CAD build for the part. Positions are in the model's coordinates, mm. Face numbers are marked on the shaded views. A direction names the side the tool comes from. Give positions to 0.01 mm unless a question says otherwise; leave off trailing zeros. Loops run counter-clockwise (first coordinate to the right, second up) from the corner with the lowest first, then second, coordinate; pieces in that order, holes last. Notation, with made-up numbers: (69.5, 53) -> (117.5, 53) arc R29 cw to (117.5, 76) -> close; hole circle Ø7 at (-13.5, 81). An arc over 180 degrees is marked (long way). Use one line per item in the form item = value.
```python
from build123d import *

# Parameters (mm, degrees)
SKETCH1_R           = 12.5
BOSS_EXTRUDE1_DEPTH = 3
SKETCH2_R           = 12
BOSS_EXTRUDE2_DEPTH = 25
SKETCH3_R           = 7.5
BOSS_EXTRUDE3_DEPTH = 12
CUT_EXTRUDE1_DEPTH  = 4
CHAMFER1_SIZE       = 1


with BuildPart() as part:
    # Sketch1 → Boss-Extrude1 (new body)
    with BuildSketch(Plane(origin=(0, 0, 0), x_dir=(1, 0, 0), z_dir=(0, 1, 0))):
        with Locations(Location((0, 0, 0), (0, 0, 270))):
            Circle(SKETCH1_R)
    extrude(amount=BOSS_EXTRUDE1_DEPTH)

    # Sketch2 → Boss-Extrude2 (add)
    with BuildSketch(Plane(origin=(0, 3, 0), x_dir=(1, 0, 0), z_dir=(0, 1, 0))):
        with Locations(Location((0, 0, 0), (0, 0, 270))):
            Circle(SKETCH2_R)
    extrude(amount=BOSS_EXTRUDE2_DEPTH)

    # Sketch3 → Boss-Extrude3 (add)
    with BuildSketch(Plane(origin=(0, 28, 0), x_dir=(1, 0, 0), z_dir=(0, 1, 0))):
        with Locations(Location((0, 0, 0), (0, 0, 270))):
            Circle(SKETCH3_R)
    extrude(amount=BOSS_EXTRUDE3_DEPTH)

    # Sketch4 → Cut-Extrude1 (cut)
    with BuildSketch(Plane(origin=(0, 0, -12), x_dir=(-1, 0, 0), z_dir=(0, 0, -1))):
        with BuildLine():
            Line((4, 23), (4, 8))
            ThreePointArc((4, 8), (0, 4), (-4, 8))
            Line((-4, 8), (-4, 23))
            ThreePointArc((-4, 23), (0, 27), (4, 23))
        make_face()
    extrude(amount=-CUT_EXTRUDE1_DEPTH, mode=Mode.SUBTRACT)

    # Chamfer1
    chamfer1_edges = [part.edges().sort_by_distance(p)[0] for p in [
        (0, 40, -7.5),
        (0, 0, -12.5),
    ]]
    chamfer(chamfer1_edges, length=CHAMFER1_SIZE)


solid = part.part
```
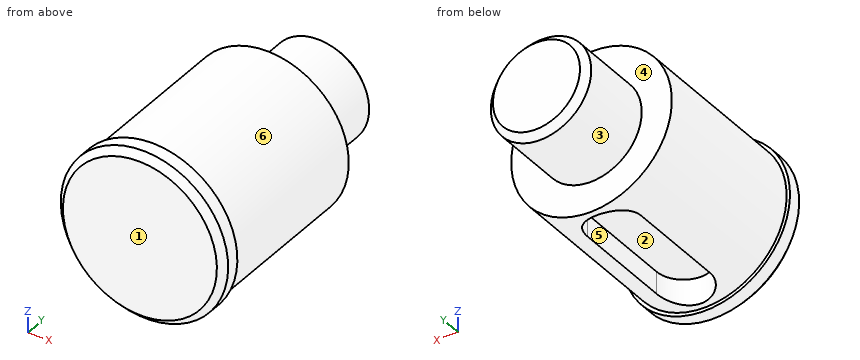
1. Cut at A-A, the plane x = 0. Write the cut outline in (y, z), then the cut area to 3 significant figures.
Result sheet:
outline = (0, -11.5) -> (1, -12.5) -> (3, -12.5) -> (3, -12) -> (4, -12) -> (4, -8) -> (27, -8) -> (27, -12) -> (28, -12) -> (28, -7.5) -> (39, -7.5) -> (40, -6.5) -> (40, 6.5) -> (39, 7.5) -> (28, 7.5) -> (28, 12) -> (3, 12) -> (3, 12.5) -> (1, 12.5) -> (0, 11.5) -> close
area = 761 mm^2
2. Cut at D-D, the plane y = 14. Write the cut outline in (x, z), then the cut area to 3 significant figures.
Result sheet:
outline = (-4, -11.31) -> (-4, -8) -> (4, -8) -> (4, -11.31) arc R12 ccw (long way) to start
area = 422 mm^2
3. Tool access for the marked faces 1, 2 and 3: list every direction of +Z, -Z, +X, -X, +Y, -Y with a clear straight run to the whole face (end or side of a thin tool).
Result sheet:
face_1 = +Z, -Z, +X, -X, -Y
face_2 = -Z
face_3 = +Y
4. Cut at B-B, the plane z = 0. Write the cut outline in (x, y), then the cut area to 3 significant figures.
Result sheet:
outline = (-12.5, 1) -> (-11.5, 0) -> (11.5, 0) -> (12.5, 1) -> (12.5, 3) -> (12, 3) -> (12, 28) -> (7.5, 28) -> (7.5, 39) -> (6.5, 40) -> (-6.5, 40) -> (-7.5, 39) -> (-7.5, 28) -> (-12, 28) -> (-12, 3) -> (-12.5, 3) -> close
area = 853 mm^2
5. Cut at C-C, the plane y = 3.5. Write the cut outline in (x, z), then the cut area to 3 significant figures.
Result sheet:
outline = circle Ø24 at (0, 0)
area = 452 mm^2
6. Mould opens along X. For the marked faces 4, 5 and 6 say: pulls with the +X half, pulls with the -X half, needs draft (parallel to the pull), parting line crosses it, or undercut.
Result sheet:
face_4 = needs draft
face_5 = undercut
face_6 = parting line crosses it
7. Drill centre lines: line 1 (Y direction, x = -5.5, z = -9); line 2 (Z direction, x = 0, y = 15.5); line 3 (X direction, y = 26, z = -9). Where is each one in solid material? Low to high.
Result sheet:
line_1 = 0 to 28
line_2 = -8 to 12
line_3 = -7.94 to -2.65, 2.65 to 7.94
8. Drop flat-ended pins along their axis: P1, Ø2.5, axis at y = 16, z = -9, coming from the -X side; P2, Ø1.5, axis at y = 15.5, z = -7.5, coming from the +X side; P3, Ø8, axis at y = 5.5, z = 5.5, coming from the +X side; P4, Ø10, axis at x = 1.5, z = -8.5, coming from the +Y side. Give the stop position or say it passes through.
Result sheet:
P1 = -9.16
P2 = 9.92
P3 = 12.27
P4 = 40
